from build123d import *

# Parameters (mm, degrees)
BASE_PLATE_12MM_DEPTH = 12
RAISED_PAD_19MM_DEPTH = 19
HUB_PROFILE_R         = 12.5
HUB_PROFILE_R_2       = 6
HUB_BOSS_34MM_DEPTH   = 34


with BuildPart() as part:
    # Base Plate Profile → Base Plate 12mm (new body)
    with BuildSketch(Plane(origin=(0, 0, 0), x_dir=(1, 0, 0), z_dir=(0, 1, 0))):
        with BuildLine():
            Line((-12.5, 35), (-22, 35))
            Line((-22, 35), (-22, 0))
            ThreePointArc((-22, 0), (-3.518993252, -21.716737473), (20.874244226, -6.947368421))
            ThreePointArc((20.874244226, -6.947368421), (26.697150325, 0.97771369), (36.055512755, 4))
            ThreePointArc((36.055512755, 4), (55.322416794, 14.463414397), (63, 35))
            Line((63, 35), (25.47250751, 35))
            Line((25.47250751, 35), (25.47250751, 19.386749889))
            ThreePointArc((25.47250751, 19.386749889), (24.121301121, 14.937756348), (20.524121628, 11.991639932))
            ThreePointArc((20.524121628, 11.991639932), (14.69106688, 7.214325266), (12.5, 0))
            ThreePointArc((12.5, 0), (0, -12.5), (-12.5, 0))
            Line((-12.5, 0), (-12.5, 35))
        make_face()
    extrude(amount=BASE_PLATE_12MM_DEPTH)

    # Raised Pad Profile → Raised Pad 19mm (add)
    with BuildSketch(Plane(origin=(0, 0, 0), x_dir=(1, 0, 0), z_dir=(0, 1, 0))):
        with BuildLine():
            ThreePointArc((20.524121628, 11.991639932), (24.121301121, 14.937756348), (25.47250751, 19.386749889))
            Line((25.47250751, 19.386749889), (25.47250751, 35))
            Line((25.47250751, 35), (0, 35))
            Line((0, 35), (0, 12.5))
            ThreePointArc((0, 12.5), (8.838834765, 8.838834765), (12.5, 0))
            ThreePointArc((12.5, 0), (14.69106688, 7.214325266), (20.524121628, 11.991639932))
        make_face()
        with BuildLine():
            Line((0, 12.5), (0, 35))
            Line((0, 35), (-12.5, 35))
            Line((-12.5, 35), (-12.5, 0))
            ThreePointArc((-12.5, 0), (-8.838834765, 8.838834765), (0, 12.5))
        make_face()
    extrude(amount=RAISED_PAD_19MM_DEPTH)

    # Hub Profile → Hub Boss 34mm (add)
    with BuildSketch(Plane(origin=(0, 0, 0), x_dir=(1, 0, 0), z_dir=(0, 1, 0))):
        Circle(HUB_PROFILE_R)
        with Locations(Location((0, 0, 0), (0, 0, 270))):
            Circle(HUB_PROFILE_R_2, mode=Mode.SUBTRACT)
    extrude(amount=HUB_BOSS_34MM_DEPTH)


solid = part.part
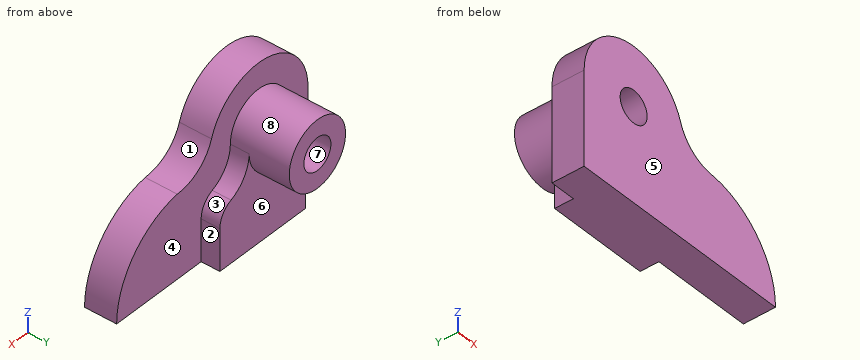
Verification items for the finished model (mm, model axes). Face numbers are marked on the shaded views. A direction names the side the tool comes from. Coordinates: 2 decimals unless noted, no trailing zeros. Write each loop counter-clockwise with the first axis right and the second up, starting at its lowest first coordinate (ties: lowest second). Pieces come first, ordered by that corner, then holes. Notation, with made-up numbers: M -12,87 L -3,87 A13 cw -3,106 Z; hole C 33.5,-18 d6. An arc over 180 degrees is marked long. Use a Markdown table: item, result.
Q1. Sectioned sample at A-A, the plane x = 0. Record the boundary of the cut face in (y, z).
Reply:
| item | result |
|---|---|
| outline | M 0,-35 L 19,-35 L 19,-12.5 L 34,-12.5 L 34,-6 L 0,-6 Z; M 0,6 L 34,6 L 34,12.5 L 12,12.5 L 12,22 L 0,22 Z |
Q2. Sectioned sample at B-B, the plane y = 16. Record the boundary of the cut face in (x, z).
Reply:
| item | result |
|---|---|
| outline | M -12.5,-35 L 25.47,-35 L 25.47,-19.39 A8 ccw 20.52,-11.99 A12.97 cw 12.5,0 A12.5 ccw -12.5,0 Z; hole C 0,0 d12 |
Q3. Sectioned sample at C-C, the plane z = 11. Record the boundary of the cut face in (x, y).
Reply:
| item | result |
|---|---|
| outline | M -19.05,0 L 19.05,0 L 19.05,12 L 5.94,12 L 5.94,34 L -5.94,34 L -5.94,12 L -19.05,12 Z |
Q4. Set-up check for the marked faces 1, 2, 3, 4 and 5: record each of +Z, -Z, +X, -X, +Y, -Y from which the full face is reachable in a straight line by a thin tool's end or side.
Reply:
| item | result |
|---|---|
| face 1 | +Z, +X, +Y, -Y |
| face 2 | +Z, -Z, +X, +Y |
| face 3 | +Z, +X, +Y |
| face 4 | +Z, +Y |
| face 5 | +Z, -Z, +X, -X, -Y |
Q5. Draft check along Z on the marked faces 6, 7 and 8. Enter one of: +Z half, -Z half, draft (parallel to the pull), parting line (faces both ways), or undercut.
Reply:
| item | result |
|---|---|
| face 6 | draft |
| face 7 | undercut |
| face 8 | parting line |
Q6. Go/stop test with flat-tipped pins: P1, Ø10, axis at y = 20, z = -16.5, coming from the -X side; P2, Ø11, axis at x = 0, z = 0, coming from the -Y side; P3, Ø3, axis at y = 6.5, z = -15.5, coming from the +X side; P4, Ø10, axis at y = 8, z = 14, coming from the -X side. Record where each tip stops, or that it passes through.
Reply:
| item | result |
|---|---|
| P1 | stops at x = -12.5 |
| P2 | passes through |
| P3 | stops at x = 57.31 |
| P4 | stops at x = -20.07 |
Q7. Thickness scan on line 1 (X direction, y = 16, z = 0); line 2 (Y direction, x = 7, z = 19); line 3 (Y direction, x = -2.5, z = -26.5). Record the ranges inside material, lowest first.
Reply:
| item | result |
|---|---|
| line 1 | x = -12.5 to -6, 6 to 12.5 |
| line 2 | y = 0 to 12 |
| line 3 | y = 0 to 19 |
Q8. Sectioned sample at D-D, the plane y = 3. Record the boundary of the cut face in (x, z), plus the area to 3 significant figures.
Reply:
| item | result |
|---|---|
| outline | M -22,-35 L 63,-35 A31.31 ccw 36.06,-4 A16 cw 20.87,6.95 A22 ccw -22,0 Z; hole C 0,0 d12 |
| area | 3,290 mm² |
